Read the model definition and answer for the solid it produces. Units are mm, in the model's axes. Coordinates: 2 decimals unless noted, no trailing zeros. Write each loop counter-clockwise with the first axis right and the second up, starting at its lowest first coordinate (ties: lowest second). Pieces come first, ordered by that corner, then holes. Notation, with made-up numbers: (-26.75, 7.5) - (11.25, 7.5) arc R24 cw to (11.25, 21.5) - close; hole circle Ø2 at (14, -32.75). An arc over 180 degrees is marked (long way). Use a Markdown table: item, result.
from build123d import *
from OCP.BRepFilletAPI import BRepFilletAPI_MakeChamfer

# Parameters (mm, degrees)
SKETCH1_W           = 40
SKETCH1_H           = 80
BOSS_EXTRUDE1_DEPTH = 2
SKETCH2_R           = 2.5
CUT_EXTRUDE1_DEPTH  = 10
CHAMFER1_SIZE       = 5
CHAMFER1_SIZE2      = 10


with BuildPart() as part:
    # Sketch1 → Boss-Extrude1 (new body)
    with BuildSketch(Plane(origin=(0, 0, 0), x_dir=(1, 0, 0), z_dir=(0, 1, 0))):
        Rectangle(SKETCH1_W, SKETCH1_H)
    extrude(amount=BOSS_EXTRUDE1_DEPTH)

    # Sketch2 → Cut-Extrude1 (cut)
    with BuildSketch(Plane.XZ):
        with Locations(Location((8, -20, 0), (0, 0, 270))):
            Circle(SKETCH2_R)
        with Locations(Location((-8, -20, 0), (0, 0, 270))):
            Circle(SKETCH2_R)
    extrude(amount=-CUT_EXTRUDE1_DEPTH, mode=Mode.SUBTRACT)

    # Chamfer1: one chamfer whose edges measure the first distance from different faces: ONE call of the kernel's chamfer builder (chamfer() names one face for all edges)
    chamfer1_edges_1 = [part.edges().sort_by_distance(p)[0] for p in [
        (20, 1, 40),
    ]]
    chamfer1_side_1 = [part.faces().sort_by_distance(p)[0] for p in [
        (0, 1, 40),
    ]]
    chamfer1_edges_2 = [part.edges().sort_by_distance(p)[0] for p in [
        (-20, 1, 40),
    ]]
    chamfer1_side_2 = [part.faces().sort_by_distance(p)[0] for p in [
        (-20, 1, 0),
    ]]
    chamfer1 = BRepFilletAPI_MakeChamfer(part.part.solid().wrapped)
    for e in chamfer1_edges_1:
        chamfer1.Add(CHAMFER1_SIZE, CHAMFER1_SIZE2, e.wrapped, chamfer1_side_1[0].wrapped)  # the first distance lies on this face
    for e in chamfer1_edges_2:
        chamfer1.Add(CHAMFER1_SIZE, CHAMFER1_SIZE2, e.wrapped, chamfer1_side_2[0].wrapped)  # the first distance lies on this face
    add(Compound.cast(chamfer1.Shape()), mode=Mode.REPLACE)


solid = part.part
(1) The mould has two halves that part along X. Classify faces 1 (the flat face through (0, 1, -40)), 2 (the flat face through (20, 1, -5)), 3 (the cylindrical face through (6.5, 1, -18)): pulls with the +X half, pulls with the -X half, needs draft (parallel to the pull), parting line crosses it, or undercut.
Report:
| item | result |
|---|---|
| face 1 | needs draft |
| face 2 | pulls with the +X half |
| face 3 | undercut |
(2) A cutting plane is placed at D-D, the plane z = 32. Write down the section's boundary in (x, y), and give its area (3 significant figures).
Report:
| item | result |
|---|---|
| outline | (-20, 0) - (19, 0) - (19, 2) - (-20, 2) - close |
| area | 78.0 mm² |
(3) A cutting plane is placed at B-B, the plane x = 8. Write down the section's boundary in (y, z), and give its area (3 significant figures).
Report:
| item | result |
|---|---|
| outline | (0, -40) - (2, -40) - (2, -22.5) - (0, -22.5) - close; (0, -17.5) - (2, -17.5) - (2, 40) - (0, 40) - close |
| area | 150 mm² |
(4) A cutting plane is placed at A-A, the plane z = -20. Write down the section's boundary in (x, y), and give its area (3 significant figures).
Report:
| item | result |
|---|---|
| outline | (-20, 0) - (-10.5, 0) - (-10.5, 2) - (-20, 2) - close; (-5.5, 0) - (5.5, 0) - (5.5, 2) - (-5.5, 2) - close; (10.5, 0) - (20, 0) - (20, 2) - (10.5, 2) - close |
| area | 60.0 mm² |
(5) A cutting plane is placed at C-C, the plane y = 0.3. Write down the section's boundary in (x, z), and give its area (3 significant figures).
Report:
| item | result |
|---|---|
| outline | (-20, -40) - (20, -40) - (20, 30) - (15, 40) - (-10, 40) - (-20, 35) - close; hole circle Ø5 at (-8, -20); hole circle Ø5 at (8, -20) |
| area | 3,110 mm² |
(6) Straight lines are drawn through the part: L1, parallel to X at y = 1.1, z = -20; L2, parallel to Z at x = -8.5, y = 0.25; L3, parallel to Z at x = 9, y = 0.7. For each, find the intervals that lie inside material, in ascending order.
Report:
| item | result |
|---|---|
| L1 | x = -20 to -10.5, -5.5 to 5.5, 10.5 to 20 |
| L2 | z = -40 to -22.45, -17.55 to 40 |
| L3 | z = -40 to -22.29, -17.71 to 40 |
